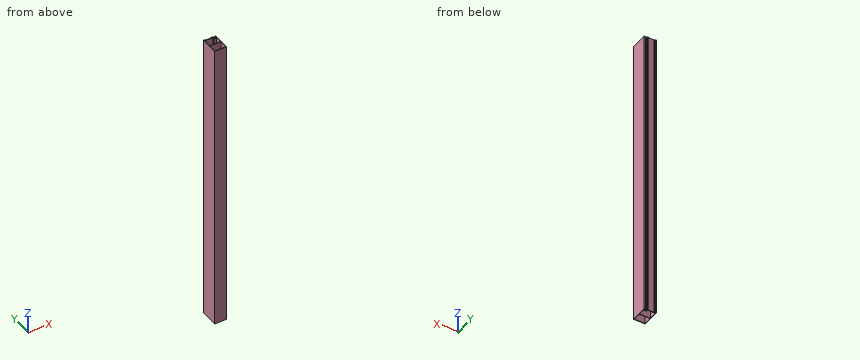
```python
from build123d import *

# Parameters (mm, degrees)
SKETCH1_W           = 39
SKETCH1_H           = 28.2
BOSS_EXTRUDE1_DEPTH = 530


with BuildPart() as part:
    # Sketch1 → Boss-Extrude1 (new, symmetric)
    with BuildSketch(Plane.XY):
        Polygon((21.5, -31), (-21.5, -31), (-21.5, 31), (-21.5, 33.5), (-19, 33.5), (-19, 31), (-15.5, 31), (-15.5, 33.5), (-14, 33.5), (-14, 31), (8, 31), (8, 33.5), (9.5, 33.5), (9.5, 31), (13.5, 31), (13.5, 29), (12.5, 29), (12.5, 24), (19.5, 24), (19.5, 29), (17.5, 29), (17.5, 31), (21.5, 31), align=None)
        Polygon((19.5, 0.8), (-19.5, 0.8), (-19.5, 29), (10.1, 29), (10.1, 22.4), (19.5, 22.4), align=None, mode=Mode.SUBTRACT)
        with Locations((0, -14.9)):
            Rectangle(SKETCH1_W, SKETCH1_H, mode=Mode.SUBTRACT)
    extrude(amount=BOSS_EXTRUDE1_DEPTH, both=True)


solid = part.part
```
Can you work these out from the model? Positions are in its coordinate system, mm. Give positions to 0.01 mm unless a question says otherwise; leave off trailing zeros. Loops run counter-clockwise (first coordinate to the right, second up) from the corner with the lowest first, then second, coordinate; pieces in that order, holes last. Notation, with made-up numbers: M -36.5,77.25 L -27.5,77.25 A31 cw -27.5,101.25 Z; hole C 51.25,-30 d10. An arc over 180 degrees is marked long. Use CSV: the item, a comma, the result in double quotes. Start each with the question number.
1. For P1, Ø11, axis at x = -4.5, z = -192, coming from the +Y side; P2, Ø10, axis at x = -11.5, y = -5, coming from the +Z side, each with a flat end and sliding along its axis, tell me the tip position at first contact or that it passes through.
2. Imagine slicing it at B-B, the plane x = -6. Write out the boundary of the cut face in (y, z).
3. Imagine slicing it at A-A, the plane z = -306. Count the separate pieces of the cut face and the enclosed holes in it, plus the area to 3 significant figures.
4. If I drill on L1, parallel to Y at x = 0.5, z = 420.5; L2, parallel to X at y = 25.5, z = -113; L3, parallel to X at y = -26, z = 364, over which ranges is the centre line in solid material (lowest first)?
Response values:
1,P1,"y = 31"
1,P2,"z = 530"
2,outline,"M -31,-530 L -29,-530 L -29,530 L -31,530 Z; M -0.8,-530 L 0.8,-530 L 0.8,530 L -0.8,530 Z; M 29,-530 L 31,-530 L 31,530 L 29,530 Z"
3,separate pieces,"1"
3,enclosed holes,"2"
3,area,"499 mm^2"
4,L1,"-31 to -29, -0.8 to 0.8, 29 to 31"
4,L2,"-21.5 to -19.5, 10.1 to 12.5, 19.5 to 21.5"
4,L3,"-21.5 to -19.5, 19.5 to 21.5"
